Build history of the part. All positions in model axes, mm. A direction names the side the tool comes from. Coordinates: 2 decimals unless noted, no trailing zeros. Loops run counter-clockwise (first coordinate to the right, second up) from the corner with the lowest first, then second, coordinate; pieces in that order, holes last.
(1) Slice it at B-B (z = 32). Give the cut face in (x, y).
(2) Wall check: L1, parallel to Y at x = 114, z = 39; L2, parallel to Y at x = 79, z = 4.5; L3, parallel to Z at x = 19, y = 24. Give the ranges that are in metal, low to high.
(3) Slice it at C-C (x = 114). Give the cut face in (y, z).
(4) Two-plate mould, pull along Y, no slides. Class faces 5 (the face through (114, 38, 26)), 6 (the face through (47, 51, 25)), 7 (the face through (80, 0, 13)): pulls with the +Y half, pulls with the -Y half, needs draft (parallel to the pull), parting line crosses it, or undercut.
(5) Flat gauge pins, fed straight in: P1, Ø3.5, axis at x = 113.5, z = 42, coming from the +Y side; P2, Ø7.5, axis at y = 88.5, z = 13.5, coming from the +X side; P3, Ø3, axis at x = 18, y = 53.5, coming from the +Z side. Where does each tip first touch, or does it go through?
(6) Tool access for faces 1 (the face through (114, 67, 34)), 2 (the face through (96, 37, 33)), 3 (the face through (132, 37, 33)), 4 (the face through (114, 10, 34)): list every direction of +Z, -Z, +X, -X, +Y, -Y with a clear straight run to the whole face (end or side of a thin tool).
(7) Slice it at A-A (y = 21). Give the cut face in (x, z).
(8) Slice it at D-D (z = 7). Give the cut face in (x, y), and give its area (3 significant figures).
from build123d import *

# Parameters (mm, degrees)
BASE_BLOCK_DEPTH   = 25
SIDE_BLOCK_DEPTH   = 25
PAD_SKETCH_W       = 36
PAD_SKETCH_H       = 76
MOUNTING_PAD_DEPTH = 9
LUG_BOSS_SKETCH_W  = 36
LUG_BOSS_SKETCH_H  = 38
LUG_BOSS_DEPTH     = 12
HOLE_SKETCH_16_R   = 8
HOLE_16_DEPTH      = 20


with BuildPart() as part:
    # Base Profile Sketch → Base Block (new body)
    with BuildSketch(Plane.XY):
        Polygon((0, 0), (162, 0), (162, 76), (25, 76), (0, 76), (0, 51), align=None)
    extrude(amount=BASE_BLOCK_DEPTH)

    # Side Block Sketch → Side Block (add)
    with BuildSketch(Plane.XY.offset(25)):
        Polygon((63, 76), (63, 101), (25, 101), (0, 76), (25, 76), align=None)
    extrude(amount=-SIDE_BLOCK_DEPTH)

    # Pad Sketch → Mounting Pad (add)
    with BuildSketch(Plane.XY.offset(25)):
        with Locations((114, 38)):
            Rectangle(PAD_SKETCH_W, PAD_SKETCH_H)
    extrude(amount=MOUNTING_PAD_DEPTH)

    # Lug Boss Sketch → Lug Boss (add)
    with BuildSketch(Plane.XY.offset(34)):
        with Locations((114, 38)):
            Rectangle(LUG_BOSS_SKETCH_W, LUG_BOSS_SKETCH_H)
    extrude(amount=LUG_BOSS_DEPTH)

    # Hole Sketch Ø16 → Hole Ø16 (cut)
    with BuildSketch(Plane.XY.offset(46)):
        with Locations((114, 38)):
            Circle(HOLE_SKETCH_16_R)
    extrude(amount=-HOLE_16_DEPTH, mode=Mode.SUBTRACT)


solid = part.part
Response values:
1. outline: (96, 0) - (132, 0) - (132, 76) - (96, 76) - close; hole circle Ø16 at (114, 38)
2. L1: y = 19 to 30, 46 to 57
2. L2: y = 0 to 76
2. L3: z = 0 to 25
3. outline: (0, 0) - (76, 0) - (76, 34) - (57, 34) - (57, 46) - (46, 46) - (46, 26) - (30, 26) - (30, 46) - (19, 46) - (19, 34) - (0, 34) - close
4. face 5: undercut
4. face 6: needs draft
4. face 7: pulls with the -Y half
5. P1: stops at y = 57
5. P2: stops at x = 63
5. P3: stops at z = 25
6. face 1: +Z, +X, -X, +Y
6. face 2: +Z, -X, +Y, -Y
6. face 3: +Z, +X, +Y, -Y
6. face 4: +Z, +X, -X, -Y
7. outline: (0, 0) - (162, 0) - (162, 25) - (132, 25) - (132, 46) - (96, 46) - (96, 25) - (0, 25) - close
8. outline: (0, 0) - (162, 0) - (162, 76) - (63, 76) - (63, 101) - (25, 101) - (0, 76) - close
8. area: 13,600 mm2
